Build history of the part. All positions in model axes, mm. A direction names the side the tool comes from. Round coordinates to 2 decimals unless told otherwise and drop trailing zeros. Order: outer loops, then holes, each group sorted by start corner. A loop starts at its lowest first (then second) coordinate and runs counter-clockwise, first axis right, second up. Notation, with made-up numbers: (48, 49.25) -> (107, 49.25) arc R15 cw to (107, 76.25) -> close; hole circle Ø7 at (16, -32.75). An arc over 180 degrees is marked (long way). Use a Markdown table: item, result. Add a question column.
Item 1: Probe L1, parallel to Y at x = -70, z = 264; L2, parallel to X at y = 38, z = 128; L3, parallel to Z at x = -67, y = -6.5. List the from-to ranges inside material, lowest first.
Item 2: Slice it at B-B, the plane x = -70. Give the cut face in (y, z).
Item 3: Slice it at A-A, the plane y = 0. Give the cut face in (x, z), plus the area to 3 significant figures.
Item 4: Two-plate mould, pull along X, no slides. Class faces 1 (the face through (-45, -1, 122)), 2 (the face through (-1, 45, 146)), 3 (the face through (-65.84, -1.72, 268.28)): released by +X, released by -X, zero draft, split by the parting line, or undercut.
Item 5: Slice it at D-D, the plane y = 26. Give the cut face in (x, z).
Item 6: Slice it at C-C, the plane z = 98.5. Give the cut face in (x, y), plus the area to 3 significant figures.
Item 7: Pin check, flat tips, straight feed: pin 1 (24 mm diameter, centred on y = -4, z = 145.5, fed in from -X); pin 2 (1 mm diameter, centred on y = -29.5, z = 195.5, fed in from +X); pin 3 (7 mm diameter, centred on x = -70, y = 0, fed in from -Z); pin 4 (1 mm diameter, centred on x = -50, y = -21.5, fed in from -Z). Stop position of each tip, or through.
Item 8: 3-axis set-ups, long thin cutter, end or side, ignore diameter. For faces 4 (the face through (-1, 1, 0)), 5 (the face through (45, -1, 122)): which of +Z, -Z, +X, -X, +Y, -Y reach the whole face in a straight line?
from build123d import *

# Parameters (mm, degrees)
SKETCH1_W            = 90
SKETCH1_H            = 90
BOSS_EXTRUDE1_DEPTH  = 288
SKETCH2_W            = 170
SKETCH2_H            = 90
BOSS_EXTRUDE2_DEPTH  = 40
CHAMFER1_SIZE        = 5
M8_CLEARANCE_HOLE1_D = 9


with BuildPart() as part:
    # Sketch1 → Boss-Extrude1 (new body)
    with BuildSketch(Plane.XY):
        Rectangle(SKETCH1_W, SKETCH1_H)
    extrude(amount=BOSS_EXTRUDE1_DEPTH)

    # Sketch2 → Boss-Extrude2 (add)
    with BuildSketch(Plane.XY.offset(288)):
        Rectangle(SKETCH2_W, SKETCH2_H)
    extrude(amount=-BOSS_EXTRUDE2_DEPTH)

    # Chamfer1
    chamfer1_edges = [part.edges().sort_by_distance(p)[0] for p in [
        (45, -45, 124),
        (-45, -45, 124),
        (-45, 45, 124),
        (45, 45, 124),
        (-85, 45, 268),
        (85, -45, 268),
        (-85, -45, 268),
        (85, 45, 268),
    ]]
    chamfer(chamfer1_edges, length=CHAMFER1_SIZE)

    # M8 Clearance Hole1 (through all)
    with Locations(Plane(origin=(0, 0, 248), x_dir=(-1, 0, 0), z_dir=(0, 0, -1))):
        with Locations((-70, 0), (70, 0)):
            Hole(M8_CLEARANCE_HOLE1_D / 2)


solid = part.part
Check sheet entries:
| question | item | result |
|---|---|---|
| 1 | L1 | -45 to -4.5, 4.5 to 45 |
| 1 | L2 | -45 to 45 |
| 1 | L3 | 248 to 288 |
| 2 | outline | (-45, 248) -> (-4.5, 248) -> (-4.5, 288) -> (-45, 288) -> close; (4.5, 248) -> (45, 248) -> (45, 288) -> (4.5, 288) -> close |
| 3 | outline | (-85, 248) -> (-74.5, 248) -> (-74.5, 288) -> (-85, 288) -> close; (-65.5, 248) -> (-45, 248) -> (-45, 0) -> (45, 0) -> (45, 248) -> (65.5, 248) -> (65.5, 288) -> (-65.5, 288) -> close; (74.5, 248) -> (85, 248) -> (85, 288) -> (74.5, 288) -> close |
| 3 | area | 28,400 mm2 |
| 4 | face 1 | released by -X |
| 4 | face 2 | zero draft |
| 4 | face 3 | undercut |
| 5 | outline | (-85, 248) -> (-45, 248) -> (-45, 0) -> (45, 0) -> (45, 248) -> (85, 248) -> (85, 288) -> (-85, 288) -> close |
| 6 | outline | (-45, -40) -> (-40, -45) -> (40, -45) -> (45, -40) -> (45, 40) -> (40, 45) -> (-40, 45) -> (-45, 40) -> close |
| 6 | area | 8,050 mm2 |
| 7 | pin 1 | x = -45 |
| 7 | pin 2 | x = 45 |
| 7 | pin 3 | through |
| 7 | pin 4 | z = 248 |
| 8 | face 4 | -Z, +X, -X, +Y, -Y |
| 8 | face 5 | -Z, +X, +Y, -Y |
